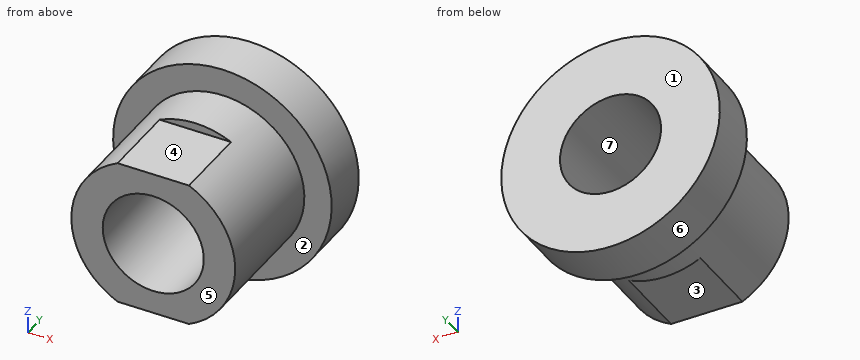
```python
from build123d import *

# Parameters (mm, degrees)
SKETCH1_R               = 20
SKETCH1_R_2             = 9
BOSS_EXTRUDE1_DEPTH     = 32
SKETCH2_R               = 25
SKETCH2_R_2             = 15
CUT_EXTRUDE1_DEPTH      = 23
CUT_EXTRUDE2_DEPTH      = 43.708313008
CUT_EXTRUDE2_DEPTH_BACK = 43.708313008
SKETCH3_W               = 7.488703297
SKETCH3_H               = 21.290197802
M20X1_5_TAPPED_HOLE1_D  = 18.5


with BuildPart() as part:
    # Sketch1 → Boss-Extrude1 (new body)
    with BuildSketch(Plane(origin=(0, 0, 0), x_dir=(1, 0, 0), z_dir=(0, 1, 0))):
        with Locations(Location((0, 0, 0), (0, 0, 270))):
            Circle(SKETCH1_R)
        with Locations(Location((0, 0, 0), (0, 0, 270))):
            Circle(SKETCH1_R_2, mode=Mode.SUBTRACT)
    extrude(amount=BOSS_EXTRUDE1_DEPTH)

    # Sketch2 → Cut-Extrude1 (cut)
    with BuildSketch(Plane.XZ):
        Circle(SKETCH2_R)
        with Locations(Location((0, 0, 0), (0, 0, 270))):
            Circle(SKETCH2_R_2, mode=Mode.SUBTRACT)
    extrude(amount=-CUT_EXTRUDE1_DEPTH, mode=Mode.SUBTRACT)

    # Sketch3 → Cut-Extrude2 (cut, two sides: drawn at the far end of the back side and taken through both)
    with BuildSketch(Plane(origin=(0, 0, 0), x_dir=(0, 0, -1), z_dir=(1, 0, 0)).offset(-CUT_EXTRUDE2_DEPTH_BACK)):
        with Locations((-17.244351649, 3.354901099)):
            Rectangle(SKETCH3_W, SKETCH3_H)
        with Locations((17.244351649, 3.354901099)):
            Rectangle(SKETCH3_W, SKETCH3_H)
    extrude(amount=CUT_EXTRUDE2_DEPTH + CUT_EXTRUDE2_DEPTH_BACK, mode=Mode.SUBTRACT)

    # M20x1.5 Tapped Hole1 (through all)
    with Locations(Plane(origin=(0, 32, 0), x_dir=(1, 0, 0), z_dir=(0, 1, 0))):
        with Locations((0, 0)):
            Hole(M20X1_5_TAPPED_HOLE1_D / 2)


solid = part.part
```
Work out the finished part from the listing and answer in its coordinate system (mm). Face numbers are marked on the shaded views. A direction names the side the tool comes from. Give positions to 0.01 mm unless a question says otherwise; leave off trailing zeros. Loops run counter-clockwise (first coordinate to the right, second up) from the corner with the lowest first, then second, coordinate; pieces in that order, holes last. Notation, with made-up numbers: (6, 26) - (48, 26) arc R9 cw to (48, 43) - close; hole circle Ø8 at (6, 23). An arc over 180 degrees is marked (long way). One line per question, with ' | ' between items.
(1) The part is cut by section B-B (y = 8). Write down the section's boundary in (x, z), then the cut area to 3 significant figures.
Recorded:
outline: (-6.54, -13.5) - (6.54, -13.5) arc R15 ccw to (6.54, 13.5) - (-6.54, 13.5) arc R15 ccw to start; hole circle Ø18.5 at (0, 0) | area: 412 mm²
(2) The part is cut by section D-D (x = -6). Write down the section's boundary in (y, z).
Recorded:
outline: (0, -13.5) - (14, -13.5) - (14, -13.75) - (23, -13.75) - (23, -19.08) - (32, -19.08) - (32, -7.04) - (0, -7.04) - close; (0, 7.04) - (32, 7.04) - (32, 19.08) - (23, 19.08) - (23, 13.75) - (14, 13.75) - (14, 13.5) - (0, 13.5) - close
(3) Straight lines are drawn through the part: probe 1 along Z at (x, y) = (0, 19); probe 2 along Z at (x, y) = (13.5, 10); probe 3 along Z at (x, y) = (-3, 11.5). For each, find the intervals that lie inside material, in ascending order.
Recorded:
probe 1: z = -15 to -9.25, 9.25 to 15 | probe 2: z = -6.54 to 6.54 | probe 3: z = -13.5 to -8.75, 8.75 to 13.5
(4) Each of these flat-tipped pins is pushed along its axis until it touches: pin 1 Ø6.5 at (x, y) = (1.5, 7) entering from +Z; pin 2 Ø4 at (x, y) = (6.5, 7.5) entering from -Z; pin 3 Ø8 at (x, y) = (7.5, 15.5) entering from +Z; pin 4 Ø6 at (x, z) = (0, -11.5) entering from -Y. Where does it stop, or does it pass through?
Recorded:
pin 1: stops at z = 13.5 | pin 2: stops at z = -13.5 | pin 3: stops at z = 14.59 | pin 4: stops at y = 0
(5) A tool of negligible diameter and unlimited length cuts with its end or side. For the marked faces 1, 2 and 3, from which of +Z, -Z, +X, -X, +Y, -Y can it reach the whole face along a straight path? Write none if from no direction.
Recorded:
face 1: +Z, -Z, +X, -X, +Y | face 2: -Y | face 3: -Z, +X, -X, -Y
(6) The mould has two halves that part along Z. Classify the marked faces 4, 5, 6 and 7: +Z half, -Z half, draft (parallel to the pull), parting line (faces both ways), or undercut.
Recorded:
face 4: +Z half | face 5: draft | face 6: parting line | face 7: undercut
(7) The part is cut by section C-C (z = 0). Write down the section's boundary in (x, y).
Recorded:
outline: (-20, 23) - (-15, 23) - (-15, 0) - (-9.25, 0) - (-9.25, 32) - (-20, 32) - close; (9.25, 0) - (15, 0) - (15, 23) - (20, 23) - (20, 32) - (9.25, 32) - close
(8) The part is cut by section A-A (x = 0). Write down the section's boundary in (y, z).
Recorded:
outline: (0, -13.5) - (14, -13.5) - (14, -15) - (23, -15) - (23, -20) - (32, -20) - (32, -9.25) - (0, -9.25) - close; (0, 9.25) - (32, 9.25) - (32, 20) - (23, 20) - (23, 15) - (14, 15) - (14, 13.5) - (0, 13.5) - close
